Check sheet for the modelled part. Datum: model origin and axes. Units: mm. Give positions to 0.01 mm unless a question says otherwise; leave off trailing zeros. Loops run counter-clockwise (first coordinate to the right, second up) from the corner with the lowest first, then second, coordinate; pieces in that order, holes last. Notation, with made-up numbers: (19, -5) -> (75, -5) arc R10 cw to (75, 0) -> close; hole circle Ø8 at (26.25, 54). An arc over 180 degrees is marked (long way). Answer as CSV lines item,"result". Start each with the question number.
(1) Gauge pin test, flat ends, axial feed: pin 1 Ø5 at (x, z) = (62, -2) entering from -Y; pin 2 Ø1.9 at (x, z) = (-1.5, -5) entering from +Y; pin 3 Ø2.5 at (y, z) = (5, -2) entering from -X. Record the tip position at first contact, or that the pin passes through.
(2) Material ranges on line 1 (X direction, y = 2.75, z = 18); line 2 (Z direction, x = -204.75, y = 5); line 3 (Y direction, x = -209, z = 18), recorded low to high. Write a range as from..to.
(3) Section check A-A on x = -103. Enter the section's corners in (y, z), plus the area to 3 significant figures.
(4) Section check B-B on x = 44. Enter the section's corners in (y, z), plus the area to 3 significant figures.
from build123d import *

# Parameters (mm, degrees)
SKETCH_1_W                   = 426
SKETCH_1_H                   = 50
EXTRUDE_1_DEPTH              = 10
HOLE_WIZARD_M4_1_AT_2_COUNT  = 2
HOLE_WIZARD_M4_1_AT_2_PITCH  = 20
HOLE_WIZARD_M3_1_D           = 3.4
HOLE_WIZARD_M3_1_CBORE_D     = 6.5
HOLE_WIZARD_M3_1_CBORE_DEPTH = 3.4
HOLE_WIZARD_M4_2_D           = 3.3
CHAMFER_1_SIZE               = 15
CHAMFER_1_SIZE2              = 190
CHAMFER_2_SIZE               = 190
CHAMFER_2_SIZE2              = 15


with BuildPart() as part:
    # 草图1 → 凸台-拉伸1 (new body)
    with BuildSketch(Plane(origin=(0, 0, 0), x_dir=(1, 0, 0), z_dir=(0, 1, 0))):
        Rectangle(SKETCH_1_W, SKETCH_1_H)
    extrude(amount=EXTRUDE_1_DEPTH)

    # 草图3 → M4 螺纹孔1 (revolve, cut)
    with BuildSketch(Plane(origin=(-213, 5, -2), x_dir=(0, 0, 1), z_dir=(0, 1, 0))):
        Polygon((0, 0), (0, 12.491420021), (1.65, 11.5), (1.65, 0), align=None)
    hole_wizard_m4_1 = revolve(axis=Axis((-219.35, 5, -2), (1, 0, 0)), mode=Mode.SUBTRACT)

    # M4 螺纹孔1 at 2: M4 螺纹孔1 ×2
    with Locations(*[(0, 0, i * HOLE_WIZARD_M4_1_AT_2_PITCH) for i in range(1, HOLE_WIZARD_M4_1_AT_2_COUNT)]):
        add(hole_wizard_m4_1, mode=Mode.SUBTRACT)

    # 镜向1: M4 螺纹孔1 across plane
    add(hole_wizard_m4_1.mirror(Plane(origin=(0, 0, 0), x_dir=(0, 0, 1), z_dir=(1, 0, 0))), mode=Mode.SUBTRACT)

    # 镜向1 copy 1 sketch → 镜向1 copy 1 (revolve, cut)
    with BuildSketch(Plane(origin=(213, 5, 18), x_dir=(0, 0, 1), z_dir=(0, 1, 0))):
        Polygon((0, 0), (0, -12.491420021), (1.65, -11.5), (1.65, 0), align=None)
    revolve(axis=Axis((219.35, 5, 18), (1, 0, 0)), mode=Mode.SUBTRACT)

    # M3 六角凹头螺钉的柱形沉头孔1 (through all)
    with Locations(Plane(origin=(0, 10, 0), x_dir=(1, 0, 0), z_dir=(0, 1, 0))):
        with Locations((10, -18), (-10, -18), (0, 5.7)):
            CounterBoreHole(HOLE_WIZARD_M3_1_D / 2, HOLE_WIZARD_M3_1_CBORE_D / 2, HOLE_WIZARD_M3_1_CBORE_DEPTH)

    # M4 螺纹孔2 (through all)
    with Locations(Plane(origin=(0, 10, 0), x_dir=(1, 0, 0), z_dir=(0, 1, 0))):
        with Locations((-38, 5), (-88, 5), (-138, 5), (-188, 5)):
            hole_wizard_m4_2 = Hole(HOLE_WIZARD_M4_2_D / 2)

    # 镜向2: M4 螺纹孔2 across plane
    add(hole_wizard_m4_2.mirror(Plane(origin=(0, 0, 0), x_dir=(0, 0, 1), z_dir=(1, 0, 0))), mode=Mode.SUBTRACT)

    # 倒角1
    chamfer_1_edges = [part.edges().sort_by_distance(p)[0] for p in [
        (213, 5, -25),
    ]]
    chamfer_1_side = [part.faces().sort_by_distance(p)[0] for p in [
        (213, 5, -0.283390906),
    ]]
    chamfer(chamfer_1_edges, length=CHAMFER_1_SIZE, length2=CHAMFER_1_SIZE2, reference=chamfer_1_side[0])

    # 倒角2
    chamfer_2_edges = [part.edges().sort_by_distance(p)[0] for p in [
        (-213, 5, -25),
    ]]
    chamfer_2_side = [part.faces().sort_by_distance(p)[0] for p in [
        (-95, 5, -25),
    ]]
    chamfer(chamfer_2_edges, length=CHAMFER_2_SIZE, length2=CHAMFER_2_SIZE2, reference=chamfer_2_side[0])


solid = part.part
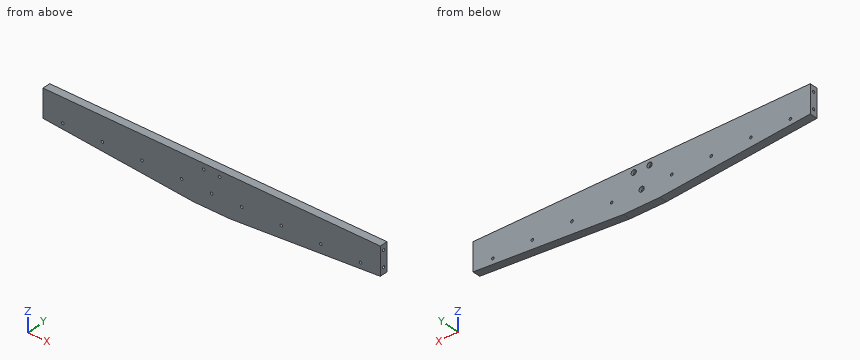
Working result:
1,pin 1,"stops at y = 0"
1,pin 2,"stops at y = 6.6"
1,pin 3,"stops at x = -201.26"
2,line 1,"x = -213..-11.7, -8.3..8.3, 11.7..213"
2,line 2,"z = -10.65..-3.65, -0.35..16.35, 19.65..25"
2,line 3,"y = 0..3.35, 6.65..10"
3,outline,"(0, -18.68) -> (10, -18.68) -> (10, 25) -> (0, 25) -> close"
3,area,"437 mm^2"
4,outline,"(0, -23.34) -> (10, -23.34) -> (10, 25) -> (0, 25) -> close"
4,area,"483 mm^2"
